The listing builds one solid part. Answer for the finished solid, in the listing's coordinates (mm). Face numbers are marked on the shaded views. Give positions to 0.01 mm unless a question says otherwise; leave off trailing zeros. Loops run counter-clockwise (first coordinate to the right, second up) from the corner with the lowest first, then second, coordinate; pieces in that order, holes last. Notation, with made-up numbers: (10, -12.75) - (62, -12.75) arc R26 cw to (62, 23.25) - close; hole circle Ø3 at (69.5, 72.25). An arc over 180 degrees is marked (long way). Answer as CSV lines item,"result". Start each with the question number.
1) For a pull along X with two mould halves and no side action, classify the marked faces 1, 2 and 3 as pulls with the +X half, pulls with the -X half, needs draft (parallel to the pull), parting line crosses it, or undercut.
2) Flat-ended cylindrical pins translate along their axes: pin 1 (6 mm diameter, centred on y = 3, z = -22, fed in from +X); pin 2 (1 mm diameter, centred on x = -27.5, y = 11.5, fed in from +Z); pin 3 (2 mm diameter, centred on x = 13.42, z = -7.75, fed in from -Y); pin 4 (6 mm diameter, centred on x = 32, z = 0, fed in from +Y). Find the tip coordinate at first contact, or state that the pin passes through.
3) Find the intervals of material crossed by line 1 along X through (y, z) = (6, 8); line 2 along X through (y, z) = (14.7, 0); line 3 along Z through (x, y) = (34, 6.75), in increasing order.
4) A cutting plane is placed at B-B (y = 8.5). Give the number of separate pieces and of enclosed holes in the cut face, and give its area (3 significant figures).
5) A cutting plane is placed at A-A (z = 0). Determine the outline of the cut face in (x, y).
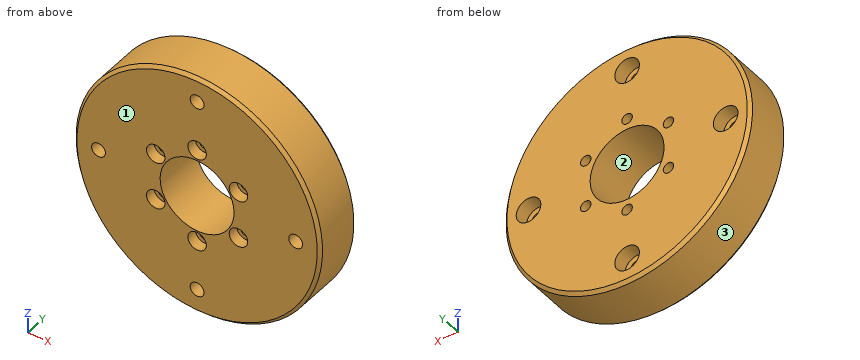
```python
from build123d import *

# Parameters (mm, degrees)
SKETCH1_R                                          = 40
SKETCH1_R_2                                        = 12
BOSS_EXTRUDE1_DEPTH                                = 16
HOLE_SIZE_BASED_HEX_SOCKET_HEAD_CAP_SC_D           = 3.4
HOLE_SIZE_BASED_HEX_SOCKET_HEAD_CAP_SC_CBORE_D     = 6
HOLE_SIZE_BASED_HEX_SOCKET_HEAD_CAP_SC_CBORE_DEPTH = 3.4
HOLE_SIZE_BASED_HEX_SOCKET_HEAD_CA_2_D             = 4.5
HOLE_SIZE_BASED_HEX_SOCKET_HEAD_CA_2_CBORE_D       = 8
HOLE_SIZE_BASED_HEX_SOCKET_HEAD_CA_2_CBORE_DEPTH   = 4.6
CIRPATTERN1_COUNT                                  = 4
CHAMFER1_SIZE                                      = 1


with BuildPart() as part:
    # Sketch1 → Boss-Extrude1 (new body)
    with BuildSketch(Plane(origin=(0, 0, 0), x_dir=(1, 0, 0), z_dir=(0, 1, 0))):
        with Locations(Location((0, 0, 0), (0, 0, 270))):
            Circle(SKETCH1_R)
        with Locations(Location((0, 0, 0), (0, 0, 270))):
            Circle(SKETCH1_R_2, mode=Mode.SUBTRACT)
    extrude(amount=BOSS_EXTRUDE1_DEPTH)

    # Hole size _based_ hex socket head cap sc (through all)
    with Locations(Plane(origin=(0, 0, 0), x_dir=(-1, 0, 0), z_dir=(0, -1, 0))):
        with Locations((0, -15.5)):
            hole_size_based_hex_socket_head_cap_sc = CounterBoreHole(HOLE_SIZE_BASED_HEX_SOCKET_HEAD_CAP_SC_D / 2, HOLE_SIZE_BASED_HEX_SOCKET_HEAD_CAP_SC_CBORE_D / 2, HOLE_SIZE_BASED_HEX_SOCKET_HEAD_CAP_SC_CBORE_DEPTH)

    # SketchPattern1: Hole size _based_ hex socket head cap sc at 5 more places
    with Locations((13.423394, 0, -23.25), (13.423394, 0, -7.75), (-13.423394, 0, -7.75), (-13.423394, 0, -23.25), (0, 0, -31)):
        add(hole_size_based_hex_socket_head_cap_sc, mode=Mode.SUBTRACT)

    # Hole size _based_ hex socket head ca 2 (through all)
    with Locations(Plane(origin=(0, 16, 0), x_dir=(1, 0, 0), z_dir=(0, 1, 0))):
        with Locations((0, 32)):
            hole_size_based_hex_socket_head_ca_2 = CounterBoreHole(HOLE_SIZE_BASED_HEX_SOCKET_HEAD_CA_2_D / 2, HOLE_SIZE_BASED_HEX_SOCKET_HEAD_CA_2_CBORE_D / 2, HOLE_SIZE_BASED_HEX_SOCKET_HEAD_CA_2_CBORE_DEPTH)

    # CirPattern1: Hole size _based_ hex socket head ca 2 ×4 about axis
    cirpattern1_axis = Axis((0, 0, 0), (0, 1, 0))
    for i in range(1, CIRPATTERN1_COUNT):
        add(hole_size_based_hex_socket_head_ca_2.rotate(cirpattern1_axis, i * 360 / CIRPATTERN1_COUNT), mode=Mode.SUBTRACT)

    # Chamfer1
    chamfer1_edges = [part.edges().sort_by_distance(p)[0] for p in [
        (0, 0, -40),
        (0, 16, -40),
    ]]
    chamfer(chamfer1_edges, length=CHAMFER1_SIZE)


solid = part.part
```
Ans:
1,face 1,"needs draft"
1,face 2,"undercut"
1,face 3,"parting line crosses it"
2,pin 1,"x = 35.2"
2,pin 2,"z = 29.51"
2,pin 3,"through"
2,pin 4,"y = 11.4"
3,line 1,"-39.19 to -15.1, -11.74 to -8.94, 8.94 to 11.74, 15.1 to 39.19"
3,line 2,"-40 to -36, -28 to -12, 12 to 28, 36 to 40"
3,line 3,"-21.07 to -1.03, 1.03 to 21.07"
4,separate pieces,"1"
4,enclosed holes,"11"
4,area,"4,460 mm2"
5,outline,"(-40, 1) - (-39, 0) - (-34.25, 0) - (-34.25, 11.4) - (-36, 11.4) - (-36, 16) - (-39, 16) - (-40, 15) - close; (-29.75, 0) - (-12, 0) - (-12, 16) - (-28, 16) - (-28, 11.4) - (-29.75, 11.4) - close; (12, 0) - (29.75, 0) - (29.75, 11.4) - (28, 11.4) - (28, 16) - (12, 16) - close; (34.25, 0) - (39, 0) - (40, 1) - (40, 15) - (39, 16) - (36, 16) - (36, 11.4) - (34.25, 11.4) - close"
